Could you check a few things on this model? Use its own coordinates, in mm. A direction names the side the tool comes from. Give positions to 0.01 mm unless a question says otherwise; leave off trailing zeros. Order: outer loops, then holes, each group sorted by start corner. A loop starts at its lowest first (then second) coordinate and runs counter-clockwise, first axis right, second up. Notation, with made-up numbers: (-4, -12.75) -> (30, -12.75) arc R17 cw to (30, 5.25) -> close; hole circle Ø5 at (12, -7). An arc over 180 degrees is marked (long way). Answer as CSV lines item,"result". Start each with the question number.
(1) I want a section at A-A (y = 16). Please give me the cut outline in (x, z).
(2) I want a section at C-C (y = 23). Please give me the cut outline in (x, z), plus the area to 3 significant figures.
(3) Will these pins go through, and if not, where does the flat tip stop? pin 1 Ø6.5 at (x, y) = (14.5, 15) entering from +Z; pin 2 Ø10 at (x, y) = (-13.5, 10) entering from +Z; pin 3 Ø8 at (x, y) = (-6, 6.5) entering from +Z; pin 4 Ø1 at (x, y) = (8.5, 13) entering from +Z.
(4) We'd pull the mould along Y, two halves only. Please class faces 4 (the face through (5, 15, -86)), 5 (the face through (-21.64, 29.1, -81.45)), 6 (the face through (3, 15, -84)): released by +Y, released by -Y, zero draft, split by the parting line, or undercut.
(5) I want a section at B-B (z = -81.75). Please give me the cut outline in (x, y).
(6) I want a section at D-D (x = -17). Please give me the cut outline in (y, z), plus the area to 3 significant figures.
(7) I need wall thicknesses on L1, parallel to X at y = 15, z = -82.75; L2, parallel to X at y = 15, z = -80.75; L3, parallel to X at y = 9, z = -81. Which ranges of each line are inside material? Lowest first, please.
(8) On a 3-axis mill with a long thin cutter (end or side, diameter ignored), from which of +Z, -Z, +X, -X, +Y, -Y can I reach the whole of each face in a straight line? I mean faces 1 (the face through (0, 2, -84)), 2 (the face through (-22.5, 15, -81)), 3 (the face through (1.75, 15, -81)). Say none if no direction works.
```python
from build123d import *

# Parameters (mm, degrees)
BOSS_EXTRUDE1_DEPTH   = 30
M8X1_0_TAPPED_HOLE1_D = 7
CUT_EXTRUDE1_DEPTH    = 39.619021662
CUT_EXTRUDE2_DEPTH    = 3.3
FILLET1_R             = 3


with BuildPart() as part:
    # Sketch1 → Boss-Extrude1 (new body)
    with BuildSketch(Plane(origin=(0, 0, 0), x_dir=(1, 0, 0), z_dir=(0, 1, 0))):
        with BuildLine():
            Line((-22.5, 76.770762664), (-22.5, 86))
            Line((-22.5, 86), (22.5, 86))
            Line((22.5, 86), (22.5, 76.770762664))
            ThreePointArc((22.5, 76.770762664), (0, 80), (-22.5, 76.770762664))
        make_face()
    extrude(amount=BOSS_EXTRUDE1_DEPTH)

    # M8x1.0 Tapped Hole1 (through all)
    with Locations(Plane(origin=(0, 0, -86), x_dir=(-1, 0, 0), z_dir=(0, 0, -1))):
        with Locations((-14.5, 15), (14.5, 15)):
            Hole(M8X1_0_TAPPED_HOLE1_D / 2)

    # Sketch4 → Cut-Extrude1 (cut, through all)
    with BuildSketch(Plane(origin=(0, 0, -86), x_dir=(-1, 0, 0), z_dir=(0, 0, -1))):
        with BuildLine():
            Line((1.75, 25), (1.75, 5))
            ThreePointArc((1.75, 5), (0, 3.25), (-1.75, 5))
            Line((-1.75, 5), (-1.75, 25))
            ThreePointArc((-1.75, 25), (0, 26.75), (1.75, 25))
        make_face()
    extrude(amount=-CUT_EXTRUDE1_DEPTH, mode=Mode.SUBTRACT)

    # Sketch5 → Cut-Extrude2 (cut)
    with BuildSketch(Plane(origin=(0, 0, -86), x_dir=(-1, 0, 0), z_dir=(0, 0, -1))):
        with BuildLine():
            Line((3, 25), (3, 5))
            ThreePointArc((3, 5), (0, 2), (-3, 5))
            Line((-3, 5), (-3, 25))
            ThreePointArc((-3, 25), (0, 28), (3, 25))
        make_face()
    extrude(amount=-CUT_EXTRUDE2_DEPTH, mode=Mode.SUBTRACT)

    # Fillet1
    fillet1_edges = [part.edges().sort_by_distance(p)[0] for p in [
        (22.5, 30, -81.385381332),
        (22.5, 0, -81.385381332),
        (-22.5, 0, -81.385381332),
        (-22.5, 30, -81.385381332),
    ]]
    fillet(fillet1_edges, radius=FILLET1_R)


solid = part.part
```
Final values:
1,outline,"(-22.5, -86) -> (-17.85, -86) -> (-17.85, -77.98) arc R80 cw to (-22.5, -76.77) -> close; (-11.15, -86) -> (-3, -86) -> (-3, -82.7) -> (-1.75, -82.7) -> (-1.75, -79.98) arc R80 cw to (-11.15, -79.22) -> close; (1.75, -82.7) -> (3, -82.7) -> (3, -86) -> (11.15, -86) -> (11.15, -79.22) arc R80 cw to (1.75, -79.98) -> close; (17.85, -86) -> (22.5, -86) -> (22.5, -76.77) arc R80 cw to (17.85, -77.98) -> close"
2,outline,"(-22.5, -86) -> (-3, -86) -> (-3, -82.7) -> (-1.75, -82.7) -> (-1.75, -79.98) arc R80 cw to (-22.5, -76.77) -> close; (1.75, -82.7) -> (3, -82.7) -> (3, -86) -> (22.5, -86) -> (22.5, -76.77) arc R80 cw to (1.75, -79.98) -> close"
2,area,"289 mm²"
3,pin 1,"through"
3,pin 2,"z = -77.83"
3,pin 3,"z = -79.37"
3,pin 4,"z = -79.49"
4,face 4,"zero draft"
4,face 5,"released by +Y"
4,face 6,"undercut"
5,outline,"(-22.5, 3) arc R3 ccw to (-19.5, 0) -> (19.5, 0) arc R3 ccw to (22.5, 3) -> (22.5, 27) arc R3 ccw to (19.5, 30) -> (-19.5, 30) arc R3 ccw to (-22.5, 27) -> close; hole circle Ø7 at (-14.5, 15); hole (-1.75, 5) arc R1.75 ccw to (1.75, 5) -> (1.75, 25) arc R1.75 ccw to (-1.75, 25) -> close; hole circle Ø7 at (14.5, 15)"
6,outline,"(0, -86) -> (12.55, -86) -> (12.55, -78.17) -> (0, -78.17) -> close; (17.45, -86) -> (30, -86) -> (30, -78.17) -> (17.45, -78.17) -> close"
6,area,"196 mm²"
7,L1,"-22.5 to -18, -11 to -3, 3 to 11, 18 to 22.5"
7,L2,"-22.5 to -18, -11 to -1.75, 1.75 to 11, 18 to 22.5"
7,L3,"-22.5 to -1.75, 1.75 to 22.5"
8,face 1,"-Z"
8,face 2,"+Z, -Z, -X, +Y, -Y"
8,face 3,"+Z, -Z"
